from build123d import *

# Parameters (mm, degrees)
HUB_TUBE_SKETCH_R   = 12.7
HUB_TUBE_SKETCH_R_2 = 7.9502
HUB_TUBE_DEPTH      = 25.6032
WEB_BOSS_DEPTH      = 12.7
FORK_EARS_SKETCH_R  = 4.7625
FORK_EARS_DEPTH     = 6.35


with BuildPart() as part:
    # Hub Tube Sketch → Hub Tube (new body)
    with BuildSketch(Plane.XY):
        Circle(HUB_TUBE_SKETCH_R)
        Circle(HUB_TUBE_SKETCH_R_2, mode=Mode.SUBTRACT)
    extrude(amount=HUB_TUBE_DEPTH)



with BuildPart() as body_2:
    # Web Boss Sketch → Web Boss (new body)
    with BuildSketch(Plane.XY):
        with BuildLine():
            Line((31.75, 9.5504), (44.45, 9.5504))
            Line((44.45, 9.5504), (44.45, 6.35))
            Line((44.45, 6.35), (31.75, 6.35))
            ThreePointArc((31.75, 6.35), (25.4, 0), (31.75, -6.35))
            Line((31.75, -6.35), (44.45, -6.35))
            Line((44.45, -6.35), (44.45, -9.5504))
            Line((44.45, -9.5504), (31.75, -9.5504))
            ThreePointArc((31.75, -9.5504), (22.1996, 0), (31.75, 9.5504))
        make_face()
    extrude(amount=WEB_BOSS_DEPTH)


with BuildPart() as part_1:
    add(part.part)

    add(body_2.part)  # Fork Ears merges body 2
    # Fork Ears Sketch → Fork Ears (add)
    with BuildSketch(Plane.XY):
        with BuildLine():
            Line((-12.7, 0), (-12.7, -14.2875))
            ThreePointArc((-12.7, -14.2875), (-13.62993597, -16.53256403), (-15.875, -17.4625))
            Line((-15.875, -17.4625), (-27.0764, -17.4625))
            ThreePointArc((-27.0764, -17.4625), (-35.0139, -25.4), (-27.0764, -33.3375))
            Line((-27.0764, -33.3375), (0, -33.3375))
            ThreePointArc((0, -33.3375), (5.621640332, -31.008940332), (7.9502, -25.3873))
            Line((7.9502, -25.3873), (7.9502, -12.7254))
            ThreePointArc((7.9502, -12.7254), (8.88013597, -10.48033597), (11.1252, -9.5504))
            Line((11.1252, -9.5504), (31.75, -9.5504))
            ThreePointArc((31.75, -9.5504), (22.1996, 0), (31.75, 9.5504))
            Line((31.75, 9.5504), (8.371371443, 9.5504))
            ThreePointArc((8.371371443, 9.5504), (5.242784693, -11.567333689), (-12.7, 0))
        make_face()
        with Locations((-27.0764, -25.4)):
            Circle(FORK_EARS_SKETCH_R, mode=Mode.SUBTRACT)
        with Locations((0, -25.3873)):
            Circle(FORK_EARS_SKETCH_R, mode=Mode.SUBTRACT)
    extrude(amount=FORK_EARS_DEPTH)


solid = part_1.part
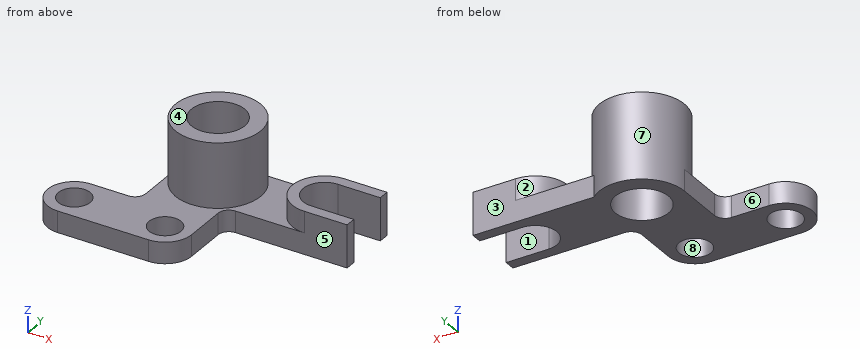
The listing builds one solid part. Answer for the finished solid, in the listing's coordinates (mm). Face numbers are marked on the shaded views. A direction names the side the tool comes from. Coordinates: 2 decimals unless noted, no trailing zeros. Loops run counter-clockwise (first coordinate to the right, second up) from the corner with the lowest first, then second, coordinate; pieces in that order, holes last.
1) Find section C-C on z = 10.5. Write down the section's boundary in (x, y), then the cut area to 3 significant figures.
2) Find section A-A on x = 34. Write down the section's boundary in (y, z), then the cut area to 3 significant figures.
3) Find section B-B on z = 3.75. Give the number of separate pieces and of enclosed holes in the cut face, then the cut area to 3 significant figures.
4) Find the intervals of material crossed by L1, parallel to Y at x = 0, z = 2; L2, parallel to Y at x = 0, z = 7.25; L3, parallel to X at y = -5, z = 6.5, in increasing order.
5) Find section D-D on y = -3.5. Write down the section's boundary in (x, z).
6) A tool of negligible diameter and unlimited length cuts with its end or side. For the marked faces 1, 2, 3, 4 and 5, from which of +Z, -Z, +X, -X, +Y, -Y can it reach the whole face along a straight path? Write none if from no direction.
7) Flat-ended cylindrical pins translate along their axes: pin 1 Ø12 at (x, z) = (25, 6) entering from +Y; pin 2 Ø5 at (y, z) = (-16, 3) entering from +X; pin 3 Ø1.5 at (y, z) = (3, 21.5) entering from +X; pin 4 Ø5.5 at (x, y) = (30.5, -0.5) entering from +Z. Find the tip coordinate at first contact, or state that the pin passes through.
8) Determine the mould class of the marked faces 6, 7 and 8 for opening direction Y: pulls with the +Y half, pulls with the -Y half, needs draft (parallel to the pull), parting line crosses it, or undercut.
Values:
1. outline: circle Ø25.4 at (0, 0); (31.75, -9.55) - (44.45, -9.55) - (44.45, -6.35) - (31.75, -6.35) arc R6.35 cw to (31.75, 6.35) - (44.45, 6.35) - (44.45, 9.55) - (31.75, 9.55) arc R9.55 ccw to start; hole circle Ø15.9 at (0, 0)
1. area: 469 mm2
2. outline: (-9.55, 0) - (-6.35, 0) - (-6.35, 12.7) - (-9.55, 12.7) - close; (6.35, 0) - (9.55, 0) - (9.55, 12.7) - (6.35, 12.7) - close
2. area: 81.3 mm2
3. separate pieces: 1
3. enclosed holes: 3
3. area: 1,360 mm2
4. L1: y = -33.34 to -30.15, -20.62 to -7.95, 7.95 to 12.7
4. L2: y = -12.7 to -7.95, 7.95 to 12.7
4. L3: x = -11.67 to -6.18, 6.18 to 11.67, 23.61 to 27.84
5. outline: (-12.7, 0) - (-7.14, 0) - (-7.14, 25.6) - (-12.21, 25.6) - (-12.21, 6.35) - (-12.7, 6.35) - close; (7.14, 0) - (26.45, 0) - (26.45, 12.7) - (22.86, 12.7) - (22.86, 6.35) - (12.21, 6.35) - (12.21, 25.6) - (7.14, 25.6) - close
6. face 1: +Z, -Z, +X
6. face 2: +Z
6. face 3: +Z, -Z, +X, +Y
6. face 4: +Z, +X, -X, +Y, -Y
6. face 5: +Z, -Z, +X, -Y
7. pin 1: stops at y = 9.55
7. pin 2: stops at x = 7.95
7. pin 3: stops at x = 12.5
7. pin 4: passes through
8. face 6: pulls with the +Y half
8. face 7: parting line crosses it
8. face 8: undercut
